Source: CAD feature listing. Evaluate the final solid. Frame: model axes, mm. A direction names the side the tool comes from. Coordinates: 2 decimals unless noted, no trailing zeros. Order: outer loops, then holes, each group sorted by start corner. A loop starts at its lowest first (then second) coordinate and runs counter-clockwise, first axis right, second up.
```python
from build123d import *

# Parameters (mm, degrees)
SKETCH1_W          = 45
SKETCH1_H          = 34
BASE_EXTRUDE_DEPTH = 16
CUT_EXTRUDE1_DEPTH = 65.381674411
FILLET1_R          = 1
FILLET2_R          = 1
CUT_EXTRUDE3_DEPTH = 65.381674411
SKETCH5_W          = 3
SKETCH5_H          = 34
CUT_EXTRUDE4_DEPTH = 65.381674411


with BuildPart() as part:
    # Sketch1 → Base-Extrude (new body)
    with BuildSketch(Plane.XY):
        with Locations((37.5, 0)):
            Rectangle(SKETCH1_W, SKETCH1_H)
    extrude(amount=BASE_EXTRUDE_DEPTH)

    # Sketch2 → Cut-Extrude1 (cut, through all)
    with BuildSketch(Plane.XY.offset(16)):
        Polygon((27, 4), (27, -4), (23, -4), (15, -12), (15, 12), (23, 4), align=None)
    extrude(amount=-CUT_EXTRUDE1_DEPTH, mode=Mode.SUBTRACT)

    # Fillet1
    fillet1_edges = [part.edges().sort_by_distance(p)[0] for p in [
        (27, 4, 8),
    ]]
    fillet(fillet1_edges, radius=FILLET1_R)

    # Fillet2
    fillet2_edges = [part.edges().sort_by_distance(p)[0] for p in [
        (27, -4, 8),
    ]]
    fillet(fillet2_edges, radius=FILLET2_R)

    # Sketch4 → Cut-Extrude3 (cut, through all)
    with BuildSketch(Plane.XY.offset(16)):
        with BuildLine():
            Line((50, 5), (50, -5))
            ThreePointArc((50, -5), (54, -9), (58, -5))
            Line((58, -5), (60, -5))
            Line((60, -5), (60, 5))
            Line((60, 5), (58, 5))
            ThreePointArc((58, 5), (54, 9), (50, 5))
        make_face()
    extrude(amount=-CUT_EXTRUDE3_DEPTH, mode=Mode.SUBTRACT)

    # Sketch5 → Cut-Extrude4 (cut, through all)
    with BuildSketch(Plane.XY.offset(16)):
        with Locations((16.5, 0)):
            Rectangle(SKETCH5_W, SKETCH5_H)
    extrude(amount=-CUT_EXTRUDE4_DEPTH, mode=Mode.SUBTRACT)


solid = part.part
```
Q1. Section query B-B on y = -6. Output: boundary loops of the cut face in (x, z), plus the area to 3 significant figures.
Solutions:
outline: (21, 0) - (50.13, 0) - (50.13, 16) - (21, 16) - close; (57.87, 0) - (60, 0) - (60, 16) - (57.87, 16) - close
area: 500 mm2
Q2. Material intervals for line 1 along Y through (x, z) = (25, 3); line 2 along X through (y, z) = (1, 4.5); line 3 along Y through (x, z) = (22, 13.25), sorted ascending.
Solutions:
line 1: y = -17 to -4, 4 to 17
line 2: x = 27 to 50
line 3: y = -17 to -5, 5 to 17
Q3. Section query A-A on x = 54. Output: boundary loops of the cut face in (y, z).
Solutions:
outline: (-17, 0) - (-9, 0) - (-9, 16) - (-17, 16) - close; (9, 0) - (17, 0) - (17, 16) - (9, 16) - close
Q4. Pull-direction query (Y, two-part tool) for faces 1 (the flat face through (27, 0, 8)), 2 (the flat face through (39, 17, 8)), 3 (the flat face through (18, -13, 8)); classes: pulls with the +Y half, pulls with the -Y half, needs draft (parallel to the pull), parting line crosses it, or undercut.
Solutions:
face 1: undercut
face 2: pulls with the +Y half
face 3: needs draft
Q5. Pin query (flat end, axial travel): P1, Ø4, axis at y = 0, z = 12.5, coming from the -X side; P2, Ø3, axis at y = -2, z = 7, coming from the +X side. Return the tip coordinate at first contact, or that it passes through.
Solutions:
P1: stops at x = 27
P2: stops at x = 50
Q6. Set-up query: faces 4 (the cylindrical face through (54, 9, 8)), 5 (the cylindrical face through (26.715, -3.699, 7.888)), 6 (the flat face through (39, 0, 16)), 7 (the flat face through (59, -5, 8)). Return all of +Z, -Z, +X, -X, +Y, -Y with unobstructed straight access to the full face (end or side cutting, diameter ignored); none if empty.
Solutions:
face 4: +Z, -Z
face 5: +Z, -Z, -X
face 6: +Z, +X, -X, +Y, -Y
face 7: +Z, -Z, +X
Q7. Section query C-C on z = 6.5. Output: boundary loops of the cut face in (x, y).
Solutions:
outline: (18, -17) - (60, -17) - (60, -5) - (58, -5) arc R4 cw to (50, -5) - (50, 5) arc R4 cw to (58, 5) - (60, 5) - (60, 17) - (18, 17) - (18, 9) - (23, 4) - (26, 4) arc R1 cw to (27, 3) - (27, -3) arc R1 cw to (26, -4) - (23, -4) - (18, -9) - close
